from build123d import *

# Parameters (mm, degrees)
SKETCH_1_R      = 12
EXTRUDE_1_DEPTH = 5
CHAMFER_1_SIZE  = 0.5


with BuildPart() as part:
    # 草图1 → 凸台-拉伸1 (new body)
    with BuildSketch(Plane(origin=(0, 0, 0), x_dir=(1, 0, 0), z_dir=(0, 1, 0))):
        with Locations(Location((0, 0, 0), (0, 0, 270))):
            Circle(SKETCH_1_R)
    extrude(amount=EXTRUDE_1_DEPTH)

    # 草图2 → M6 六角凹锥坑螺钉的锥形沉头孔1 (revolve, cut)
    with BuildSketch(Plane(origin=(0, 5, 0), x_dir=(0, 0, 1), z_dir=(1, 0, 0))):
        Polygon((0, 0), (0, 5), (3.3, 5), (3.3, 3.42), (6.72, 0), align=None)
    revolve(axis=Axis((0, 11.35, 0), (0, -1, 0)), mode=Mode.SUBTRACT)

    # 倒角1
    chamfer_1_edges = [part.edges().sort_by_distance(p)[0] for p in [
        (0, 0, -12),
        (0, 5, -12),
    ]]
    chamfer(chamfer_1_edges, length=CHAMFER_1_SIZE)


solid = part.part
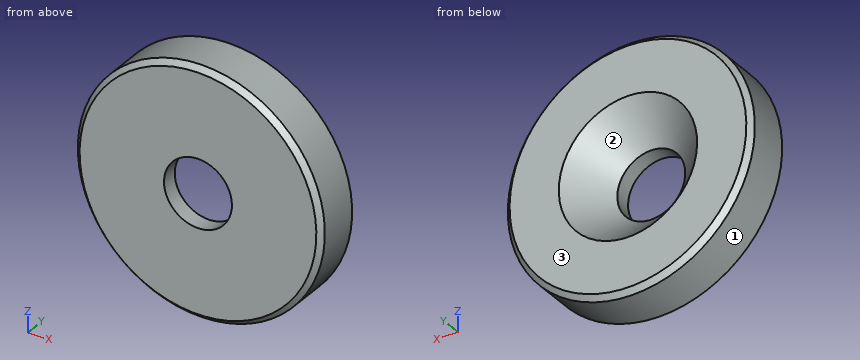
Read the model definition and answer for the solid it produces. Units are mm, in the model's axes. Face numbers are marked on the shaded views. Round coordinates to 2 decimals unless told otherwise and drop trailing zeros. Order: outer loops, then holes, each group sorted by start corner. A loop starts at its lowest first (then second) coordinate and runs counter-clockwise, first axis right, second up.
1) Straight lines are drawn through the part: L1, parallel to X at y = 0.8, z = 0; L2, parallel to X at y = 3.95, z = -5; L3, parallel to Z at x = -2.5, y = 1.7. For each, find the intervals that lie inside material, in ascending order.
2) Flat-ended cylindrical pins translate along their axes: pin 1 (1 mm diameter, centred on x = -5.5, z = 3.5, fed in from +Y); pin 2 (1.5 mm diameter, centred on y = 1, z = -2, fed in from +X). Find the tip coordinate at first contact, or state that the pin passes through.
3) The mould has two halves that part along Z. Classify the marked faces 1, 2 and 3: released by +Z, released by -Z, zero draft, split by the parting line, or undercut.
4) The part is cut by section C-C on y = 4.2. Write down the section's boundary in (x, z).
5) The part is cut by section A-A on x = 0. Write down the section's boundary in (y, z), plus the area to 3 significant figures.
6) The part is cut by section B-B on z = 0. Write down the section's boundary in (x, y), plus the area to 3 significant figures.
7) The part is cut by section D-D on y = 2.95. Write down the section's boundary in (x, z).
Resolved:
1. L1: x = -12 to -3.3, 3.3 to 12
1. L2: x = -10.91 to -2.67, 2.67 to 10.91
1. L3: z = -11.74 to -2.33, 2.33 to 11.74
2. pin 1: stops at y = 5
2. pin 2: stops at x = 11.93
3. face 1: split by the parting line
3. face 2: undercut
3. face 3: zero draft
4. outline: circle Ø24 at (0, 0); hole circle Ø11.84 at (0, 0)
5. outline: (0, -11.5) - (0.5, -12) - (4.5, -12) - (5, -11.5) - (5, -6.72) - (1.58, -3.3) - (0, -3.3) - close; (0, 3.3) - (1.58, 3.3) - (5, 6.72) - (5, 11.5) - (4.5, 12) - (0.5, 12) - (0, 11.5) - close
5. area: 74.8 mm2
6. outline: (-12, 0.5) - (-11.5, 0) - (-3.3, 0) - (-3.3, 1.58) - (-6.72, 5) - (-11.5, 5) - (-12, 4.5) - close; (3.3, 0) - (11.5, 0) - (12, 0.5) - (12, 4.5) - (11.5, 5) - (6.72, 5) - (3.3, 1.58) - close
6. area: 74.8 mm2
7. outline: circle Ø24 at (0, 0); hole circle Ø9.34 at (0, 0)
